Design review of the part built by this model. Coordinates are the model's own, in mm. A direction names the side the tool comes from. Round coordinates to 2 decimals unless told otherwise and drop trailing zeros. Order: outer loops, then holes, each group sorted by start corner. A loop starts at its lowest first (then second) coordinate and runs counter-clockwise, first axis right, second up. Notation, with made-up numbers: M 75.25,-6.5 L 102.25,-6.5 A24 cw 102.25,4.5 Z; hole C 37.5,-35.75 d5. An arc over 180 degrees is marked long. Write each question's results on one line, items separated by ' | '. Start each with the question number.
Item 1: Take a section at B-B, the plane y = -5.25. Write out the cut boundary in (x, z).
Item 2: Take a section at D-D, the plane y = -0.5. Write out the cut boundary in (x, z).
Item 3: Take a section at C-C, the plane x = 9. Write out the cut boundary in (y, z).
Item 4: Machinability: for faces 1 (the flat face through (5, -7, -30)), 2 (the flat face through (30, 4, 21)), 3 (the flat face through (17, -1.5, -15)), 4 (the flat face through (24, -7, -23)), 5 (the flat face through (4, 4, 21)), which of the approach directions +Z, -Z, +X, -X, +Y, -Y give a long, thin tool a straight path to every point of the face, cutting with its end or side? Answer none if there is none.
Item 5: Wall thickness on line 1 (X direction, y = -2.25, z = -18); line 2 (X direction, y = 5, z = 27.5); line 3 (Z direction, x = 10, y = 5.5): over which ranges is each line inside the solid? List them lowest first. Write a range as [from, to].
Item 6: Clearance check with flat-ended pins moving along their axes: pin 1 (5.5 mm diameter, centred on y = -6.5, z = -21, fed in from -X); pin 2 (3 mm diameter, centred on x = 6.5, y = 2.5, fed in from -Z); pin 3 (7 mm diameter, centred on x = 16, z = -12.5, fed in from +Y). State where each tip first meets the part, or that it passes through.
Item 7: Take a section at A-A, the plane z = -24. Write out the cut boundary in (x, y), plus the area to 3 significant figures.
```python
from build123d import *

# Parameters (mm, degrees)
BLOCK_PROFILE_SKETCH_W       = 60
BLOCK_PROFILE_SKETCH_H       = 25
BASE_BLOCK_DEPTH             = 34
STEP_CUT_PROFILE_SKETCH_W    = 24
STEP_CUT_PROFILE_SKETCH_H    = 14
STEPPED_THROUGH_CUT_DEPTH    = 34
NOTCH_PROFILE_SKETCH_W       = 14
NOTCH_PROFILE_SKETCH_H       = 13
SIDE_NOTCH_THROUGH_CUT_DEPTH = 34
SLOT_18X8_DEPTH_8_DEPTH      = 8
ARCH_RELIEF_CUT_DEPTH        = 8


with BuildPart() as part:
    # Block Profile Sketch → Base Block (new body)
    with BuildSketch(Plane(origin=(0, 0, 0), x_dir=(0, 0, -1), z_dir=(1, 0, 0))):
        Rectangle(BLOCK_PROFILE_SKETCH_W, BLOCK_PROFILE_SKETCH_H)
    extrude(amount=BASE_BLOCK_DEPTH)

    # Step Cut Profile Sketch → Stepped Through Cut (cut)
    with BuildSketch(Plane(origin=(34, 0, 0), x_dir=(0, 0, -1), z_dir=(1, 0, 0))):
        with Locations((18, 5.5)):
            Rectangle(STEP_CUT_PROFILE_SKETCH_W, STEP_CUT_PROFILE_SKETCH_H)
        with BuildLine():
            Line((-22, -12.5), (-2, -12.5))
            ThreePointArc((-2, -12.5), (-12, -2.5), (-22, -12.5))
        make_face()
    extrude(amount=-STEPPED_THROUGH_CUT_DEPTH, mode=Mode.SUBTRACT)

    # Notch Profile Sketch → Side Notch Through Cut (cut)
    with BuildSketch(Plane(origin=(0, 12.5, 0), x_dir=(1, 0, 0), z_dir=(0, 1, 0))):
        with Locations((17, 23.5)):
            Rectangle(NOTCH_PROFILE_SKETCH_W, NOTCH_PROFILE_SKETCH_H)
    extrude(amount=-SIDE_NOTCH_THROUGH_CUT_DEPTH, mode=Mode.SUBTRACT)

    # Slot Sketch → Slot 18x8 Depth 8 (cut)
    with BuildSketch(Plane(origin=(34, 0, 0), x_dir=(0, 0, -1), z_dir=(1, 0, 0))):
        Polygon((-30, 12.5), (-30, -4.5), (-12, 12.5), align=None)
    extrude(amount=-SLOT_18X8_DEPTH_8_DEPTH, mode=Mode.SUBTRACT)

    # Arch Relief Sketch → Arch Relief Cut (cut)
    with BuildSketch(Plane.ZY):
        Polygon((12, 12.5), (30, -4.5), (30, 12.5), align=None)
    extrude(amount=-ARCH_RELIEF_CUT_DEPTH, mode=Mode.SUBTRACT)


solid = part.part
```
Results list:
1) outline: M 0,-30 L 10,-30 L 10,-17 L 24,-17 L 24,-30 L 34,-30 L 34,5.11 L 0,5.11 Z; M 0,18.89 L 34,18.89 L 34,30 L 0,30 Z
2) outline: M 0,-6 L 34,-6 L 34,25.76 L 26,25.76 L 26,30 L 8,30 L 8,25.76 L 0,25.76 Z
3) outline: M -12.5,-30 L -1.5,-30 L -1.5,-6 L 12.5,-6 L 12.5,30 L -12.5,30 L -12.5,22 A10 cw -12.5,2 Z
4) face 1: -Z, +X, -X, +Y, -Y | face 2: +Z, +X, +Y | face 3: -Z, +X, -X, +Y | face 4: -Z, +Y, -Y | face 5: +Z, -X, +Y
5) line 1: [0, 10], [24, 34] | line 2: [8, 26] | line 3: [-6, 30]
6) pin 1: x = 0 | pin 2: z = -6 | pin 3: y = -1.5
7) outline: M 0,-12.5 L 10,-12.5 L 10,-1.5 L 0,-1.5 Z; M 24,-12.5 L 34,-12.5 L 34,-1.5 L 24,-1.5 Z | area: 220 mm²
